Input: part model. Units: mm. Frame: model coordinates. A direction names the side the tool comes from. Give positions to 0.01 mm unless a question says otherwise; leave off trailing zeros. Loops run counter-clockwise (first coordinate to the right, second up) from the corner with the lowest first, then second, coordinate; pieces in that order, holes last. Notation, with made-up numbers: (-32.5, -16) - (-12.5, -16) arc R8 ccw to (-12.5, -8) - close; hole circle Ø6 at (58, -17.75). An arc over 180 degrees is marked (long way). Answer as a JSON object with one key per item and string values.
from build123d import *

# Parameters (mm, degrees)
MAIN_BLOCK_DEPTH          = 82
SIDE_LUG_PROFILE_R        = 30
SIDE_LUG_PROFILE_R_2      = 10
SIDE_LUG_BOSS_DEPTH       = 45
GUSSET_BOSS_DEPTH         = 30
MOUNTING_TAB_PROFILE_W    = 70
MOUNTING_TAB_PROFILE_H    = 60
MOUNTING_TAB_DEPTH        = 25
TAB_EYE_PROFILE_R         = 20
TAB_EYE_BOSS_DEPTH        = 25
TAB_RING_PROFILES_R       = 15
TAB_RING_PROFILES_R_2     = 10
TAB_BOSS_RINGS_DEPTH      = 10
SIDE_HUB_RING_PROFILE_R   = 15
SIDE_HUB_RING_PROFILE_R_2 = 10
SIDE_HUB_RING_DEPTH       = 5
TOP_HUB_RING_PROFILE_R    = 15
TOP_HUB_RING_PROFILE_R_2  = 10
TOP_HUB_RING_DEPTH        = 15
TAB_SLOT_CUT_DEPTH        = 15


with BuildPart() as part:
    # Main Block Profile → Main Block (new body)
    with BuildSketch(Plane.XY):
        Polygon((0, 0), (25, 0), (25, 20), (55, 20), (55, 0), (80, 0), (80, 85), (0, 85), align=None)
    extrude(amount=MAIN_BLOCK_DEPTH)



with BuildPart() as body_2:
    # Side Lug Profile → Side Lug Boss (new body)
    with BuildSketch(Plane(origin=(0, 0, 0), x_dir=(1, 0, 0), z_dir=(0, 1, 0))):
        with Locations(Location((-60, -41, 0), (0, 0, 90))):
            Circle(SIDE_LUG_PROFILE_R)
        with Locations(Location((-60, -41, 0), (0, 0, 90))):
            Circle(SIDE_LUG_PROFILE_R_2, mode=Mode.SUBTRACT)
    extrude(amount=SIDE_LUG_BOSS_DEPTH)


with BuildPart() as part_1:
    add(part.part)

    add(body_2.part)  # Gusset Boss merges body 2
    # Gusset Profile → Gusset Boss (add)
    with BuildSketch(Plane(origin=(0, 0, 0), x_dir=(1, 0, 0), z_dir=(0, 1, 0))):
        with BuildLine():
            Line((0, 0), (-60, -11))
            ThreePointArc((-60, -11), (-30, -41), (-60, -71))
            Line((-60, -71), (0, -82))
            Line((0, -82), (0, 0))
        make_face()
    extrude(amount=GUSSET_BOSS_DEPTH)

    # Mounting Tab Profile → Mounting Tab (add)
    with BuildSketch(Plane(origin=(0, 0, 0), x_dir=(1, 0, 0), z_dir=(0, 1, 0))):
        with Locations((115, -41)):
            Rectangle(MOUNTING_TAB_PROFILE_W, MOUNTING_TAB_PROFILE_H)
    extrude(amount=MOUNTING_TAB_DEPTH)

    # Tab Eye Profile → Tab Eye Boss (add)
    with BuildSketch(Plane(origin=(0, 25, 0), x_dir=(1, 0, 0), z_dir=(0, 1, 0))):
        with Locations((150, -11)):
            Circle(TAB_EYE_PROFILE_R)
        with Locations((150, -71)):
            Circle(TAB_EYE_PROFILE_R)
    extrude(amount=-TAB_EYE_BOSS_DEPTH)

    # Tab Ring Profiles → Tab Boss Rings (add)
    # profile 1 of 2: a face of its own
    with BuildSketch(Plane(origin=(0, 25, 0), x_dir=(1, 0, 0), z_dir=(0, 1, 0))):
        with Locations(Location((150, -11, 0), (0, 0, 90))):
            Circle(TAB_RING_PROFILES_R)
        with Locations(Location((150, -11, 0), (0, 0, 270))):
            Circle(TAB_RING_PROFILES_R_2, mode=Mode.SUBTRACT)
    # profile 2 of 2: a face of its own
    with BuildSketch(Plane(origin=(0, 25, 0), x_dir=(1, 0, 0), z_dir=(0, 1, 0))):
        with Locations(Location((150, -71, 0), (0, 0, 90))):
            Circle(TAB_RING_PROFILES_R)
        with Locations(Location((150, -71, 0), (0, 0, 270))):
            Circle(TAB_RING_PROFILES_R_2, mode=Mode.SUBTRACT)
    extrude(amount=TAB_BOSS_RINGS_DEPTH)

    # Side Hub Ring Profile → Side Hub Ring (add)
    with BuildSketch(Plane(origin=(0, 85, 0), x_dir=(1, 0, 0), z_dir=(0, 1, 0))):
        with Locations((40, -41)):
            Circle(SIDE_HUB_RING_PROFILE_R)
        with Locations(Location((40, -41, 0), (0, 0, 180))):
            Circle(SIDE_HUB_RING_PROFILE_R_2, mode=Mode.SUBTRACT)
    extrude(amount=SIDE_HUB_RING_DEPTH)

    # Top Hub Ring Profile → Top Hub Ring (add)
    with BuildSketch(Plane.XY.offset(82)):
        with Locations((40, 57.5)):
            Circle(TOP_HUB_RING_PROFILE_R)
        with Locations((40, 57.5)):
            Circle(TOP_HUB_RING_PROFILE_R_2, mode=Mode.SUBTRACT)
    extrude(amount=TOP_HUB_RING_DEPTH)

    # Tab Slot Profile → Tab Slot Cut (cut)
    with BuildSketch(Plane(origin=(0, 25, 0), x_dir=(1, 0, 0), z_dir=(0, 1, 0))):
        Polygon((150, -41), (150, -36), (100, -36), (100, -46), (150, -46), align=None)
    extrude(amount=-TAB_SLOT_CUT_DEPTH, mode=Mode.SUBTRACT)


solid = part_1.part
Item 1: Cut plane D-D (y = 57.5). Return loops of the section in (x, z), then the cut area to 3 significant figures.
Geometry check:
{"outline": "(0, 0) - (80, 0) - (80, 82) - (55, 82) - (55, 97) - (50, 97) - (50, 82) - (30, 82) - (30, 97) - (25, 97) - (25, 82) - (0, 82) - close", "area": "6,710 mm2"}
Item 2: Access query for faces 5 (the face through (-89.745, 27.185, 44.905)), 6 (the face through (160, 35, 8)), 7 (the face through (39, 43, 0)), 8 (the face through (125, 10, 41)). Directions: +Z, -Z, +X, -X, +Y, -Y. A direction counts if a zero-diameter tool reaches every point of the face in a straight line with its end or side. Return the directions, or none.
Geometry check:
{"face 5": "+Y", "face 6": "+Z, -Z, +X, +Y", "face 7": "-Z, -X, +Y, -Y", "face 8": "+X, +Y"}
Item 3: Cut plane A-A (y = 37.5). Return loops of the section in (x, z), then the cut area to 3 significant figures.
Geometry check:
{"outline": "circle Ø60 at (-60, 41); (0, 0) - (80, 0) - (80, 82) - (0, 82) - close; hole circle Ø20 at (-60, 41)", "area": "9,070 mm2"}
Item 4: Cut plane C-C (z = 66). Return loops of the section in (x, y).
Geometry check:
{"outline": "(-76.58, 0) - (25, 0) - (25, 20) - (55, 20) - (55, 0) - (169.36, 0) - (169.36, 25) - (164.14, 25) - (164.14, 35) - (158.66, 35) - (158.66, 25) - (141.34, 25) - (141.34, 35) - (135.86, 35) - (135.86, 25) - (80, 25) - (80, 85) - (0, 85) - (0, 30) - (-43.42, 30) - (-43.42, 45) - (-76.58, 45) - close"}
Item 5: Cut plane B-B (x = 40). Return loops of the section in (y, z), then the cut area to 3 significant figures.
Geometry check:
{"outline": "(20, 0) - (85, 0) - (85, 26) - (90, 26) - (90, 31) - (85, 31) - (85, 51) - (90, 51) - (90, 56) - (85, 56) - (85, 82) - (72.5, 82) - (72.5, 97) - (67.5, 97) - (67.5, 82) - (47.5, 82) - (47.5, 97) - (42.5, 97) - (42.5, 82) - (20, 82) - close", "area": "5,530 mm2"}
Item 6: Mould query, pull axis X, two halves, no side actions, for faces 1 (the face through (150, 9.5, 41.1)), 2 (the face through (28.944, 87.465, 30.862)), 3 (the face through (125, 18, 36)), 4 (the face through (40, 58, 82)). Classes: released by +X, released by -X, zero draft, split by the parting line, or undercut.
Geometry check:
{"face 1": "released by +X", "face 2": "split by the parting line", "face 3": "zero draft", "face 4": "undercut"}
Item 7: Contact query for flat-ended pins moving along their axis: P1, Ø12, axis at y = 63.5, z = 8.5, coming from the -X side; P2, Ø6, axis at y = 46.5, z = 58.5, coming from the -X side; P3, Ø10, axis at x = 44, y = 59.5, coming from the +Z side. Output: stop coordinate, or through.
Geometry check:
{"P1": "stops at x = 0", "P2": "stops at x = -86.04", "P3": "stops at z = 82"}
Item 8: Material intervals for line 1 (Y direction, x = 40, z = 92.75); line 2 (Z direction, x = 40, y = 88.5); line 3 (Z direction, x = -60, y = 10), sorted ascending. Write a range as [from, to].
Geometry check:
{"line 1": "y = [42.5, 47.5], [67.5, 72.5]", "line 2": "z = [26, 31], [51, 56]", "line 3": "z = [11, 31], [51, 71]"}
